```python
from build123d import *

# Parameters (mm, degrees)
SKETCH_2_R          = 60
EXTRUDE_1_DEPTH     = 50
SKETCH_1_R          = 15
CUT_EXTRUDE_1_DEPTH = 30
EXTRUDE_2_DEPTH     = 20
SKETCH_5_W          = 10
SKETCH_5_H          = 6.88474508
CUT_EXTRUDE_2_DEPTH = 15


with BuildPart() as part:
    # 草图2 → 凸台-拉伸1 (new body)
    with BuildSketch(Plane.XY):
        Circle(SKETCH_2_R)
    extrude(amount=EXTRUDE_1_DEPTH)

    # 草图1 → 切除-拉伸1 (cut)
    with BuildSketch(Plane.XY):
        Circle(SKETCH_1_R)
    extrude(amount=CUT_EXTRUDE_1_DEPTH, mode=Mode.SUBTRACT)

    # 草图3 → 凸台-拉伸2 (add)
    with BuildSketch(Plane.XY.offset(50)):
        with BuildLine():
            Line((42.811529494, 42.037756153), (31.47114317, 35.490381057))
            Line((31.47114317, 35.490381057), (46.47114317, 9.509618943))
            Line((46.47114317, 9.509618943), (57.811529494, 16.05699404))
            ThreePointArc((57.811529494, 16.05699404), (51.961524227, 30), (42.811529494, 42.037756153))
        make_face()
        with BuildLine():
            Line((-15, 58.094750193), (-15, 45))
            Line((-15, 45), (15, 45))
            Line((15, 45), (15, 58.094750193))
            ThreePointArc((15, 58.094750193), (0, 60), (-15, 58.094750193))
        make_face()
        with BuildLine():
            Line((57.811529494, -16.05699404), (46.47114317, -9.509618943))
            Line((46.47114317, -9.509618943), (31.47114317, -35.490381057))
            Line((31.47114317, -35.490381057), (42.811529494, -42.037756153))
            ThreePointArc((42.811529494, -42.037756153), (51.961524227, -30), (57.811529494, -16.05699404))
        make_face()
        with BuildLine():
            Line((15, -58.094750193), (15, -45))
            Line((15, -45), (-15, -45))
            Line((-15, -45), (-15, -58.094750193))
            ThreePointArc((-15, -58.094750193), (0, -60), (15, -58.094750193))
        make_face()
        with BuildLine():
            Line((-42.811529494, -42.037756153), (-31.47114317, -35.490381057))
            Line((-31.47114317, -35.490381057), (-46.47114317, -9.509618943))
            Line((-46.47114317, -9.509618943), (-57.811529494, -16.05699404))
            ThreePointArc((-57.811529494, -16.05699404), (-51.961524227, -30), (-42.811529494, -42.037756153))
        make_face()
        with BuildLine():
            Line((-57.811529494, 16.05699404), (-46.47114317, 9.509618943))
            Line((-46.47114317, 9.509618943), (-31.47114317, 35.490381057))
            Line((-31.47114317, 35.490381057), (-42.811529494, 42.037756153))
            ThreePointArc((-42.811529494, 42.037756153), (-51.961524227, 30), (-57.811529494, 16.05699404))
        make_face()
    extrude(amount=EXTRUDE_2_DEPTH)

    # 草图5 → 切除-拉伸2 (cut)
    with BuildSketch(Plane(origin=(0, 0, 0), x_dir=(-1, 0, 0), z_dir=(0, 0, -1))):
        with Locations((0, 13.55762746)):
            Rectangle(SKETCH_5_W, SKETCH_5_H)
    extrude(amount=-CUT_EXTRUDE_2_DEPTH, mode=Mode.SUBTRACT)


solid = part.part
```
Here's how the part is built. I have some questions about the finished solid (model axes, mm). A direction names the side the tool comes from. Coordinates: 2 decimals unless noted, no trailing zeros. Write each loop counter-clockwise with the first axis right and the second up, starting at its lowest first coordinate (ties: lowest second). Pieces come first, ordered by that corner, then holes. Notation, with made-up numbers: (35.5, 18) - (77.5, 18) arc R31 ccw to (77.5, 43) - close; hole circle Ø9 at (-11.75, 9.25). An arc over 180 degrees is marked (long way). One line per item, written item: value.
1) We'd pull the mould along X, two halves only. Please class faces 1 (the flat face through (44, -26, 70)), 2 (the flat face through (-52.22, 12.83, 59.86)), 3 (the flat face through (39.076, -22.318, 59.86)): pulls with the +X half, pulls with the -X half, needs draft (parallel to the pull), parting line crosses it, or undercut.
Model answer:
face 1: needs draft
face 2: pulls with the -X half
face 3: undercut
2) On a 3-axis mill with a long thin cutter (end or side, diameter ignored), from which of +Z, -Z, +X, -X, +Y, -Y can I reach the whole of each face in a straight line? I mean faces 4 (the flat face through (-37.2, -38.8, 59.9)), 5 (the flat face through (-37.062, 38.718, 59.86)), 6 (the flat face through (0, 16, 15)). Say none if no direction works.
Model answer:
face 4: +Z, -Y
face 5: +Z, +Y
face 6: -Z
3) I need wall thicknesses on line 1 along X through (y, z) = (0, 18); line 2 along Z through (x, y) = (-30, 1.5). Which ranges of each line are inside material? Lowest first, please.
Model answer:
line 1: x = -60 to -15, 15 to 60
line 2: z = 0 to 50
4) Suppose I cut it at B-B on y = 0. Write out the boundary of the cut face in (x, z), and give its area (3 significant figures).
Model answer:
outline: (-60, 0) - (-15, 0) - (-15, 30) - (15, 30) - (15, 0) - (60, 0) - (60, 50) - (-60, 50) - close
area: 5,100 mm²
5) I'm going to push flat-ended pins straight in: P1, Ø2, axis at x = 40, z = 35.5, coming from the +Y side; P2, Ø4, axis at x = -32.5, z = 22.5, coming from the +Y side; P3, Ø10, axis at y = -26, z = 54.5, coming from the +X side (3 decimals). Where does each tip first touch, or does it pass through?
Model answer:
P1: stops at y = 45.6
P2: stops at y = 51.67
P3: stops at x = 56.205
6) Suppose I cut it at A-A on z = 66. Write out the boundary of the cut face in (x, y), and give its area (3 significant figures).
Model answer:
outline: (-57.81, -16.06) arc R60 ccw to (-42.81, -42.04) - (-31.47, -35.49) - (-46.47, -9.51) - close; (-57.81, 16.06) - (-46.47, 9.51) - (-31.47, 35.49) - (-42.81, 42.04) arc R60 ccw to start; (-15, -58.09) arc R60 ccw to (15, -58.09) - (15, -45) - (-15, -45) - close; (-15, 45) - (15, 45) - (15, 58.09) arc R60 ccw to (-15, 58.09) - close; (31.47, -35.49) - (42.81, -42.04) arc R60 ccw to (57.81, -16.06) - (46.47, -9.51) - close; (31.47, 35.49) - (46.47, 9.51) - (57.81, 16.06) arc R60 ccw to (42.81, 42.04) - close
area: 2,590 mm²
7) Suppose I cut it at C-C on z = 25. Write out the boundary of the cut face in (x, y).
Model answer:
outline: circle Ø120 at (0, 0); hole circle Ø30 at (0, 0)
8) Suppose I cut it at D-D on x = 0. Write out the boundary of the cut face in (y, z).
Model answer:
outline: (-60, 0) - (-15, 0) - (-15, 30) - (15, 30) - (15, 15) - (17, 15) - (17, 0) - (60, 0) - (60, 70) - (45, 70) - (45, 50) - (-45, 50) - (-45, 70) - (-60, 70) - close
